Check sheet for the modelled part. Datum: model origin and axes. Units: mm. Face numbers are marked on the shaded views. A direction names the side the tool comes from. Round coordinates to 2 decimals unless told otherwise and drop trailing zeros. Write each loop counter-clockwise with the first axis right and the second up, starting at its lowest first coordinate (ties: lowest second). Pieces come first, ordered by that corner, then holes. Notation, with made-up numbers: (-4.75, 17) - (36.25, 17) arc R15 ccw to (36.25, 22) - close; hole circle Ø11 at (11.5, -11). An arc over 180 degrees is marked (long way). Use one line per item in the form item = value. Start each with the question number.
1) Draft check along X on the marked faces 3, 4 and 5. Enter one of: +X half, -X half, draft (parallel to the pull), parting line (faces both ways), or undercut.
2) Scan lines: probe 1 along Y at (x, z) = (0, 3.95); probe 2 along X at (y, z) = (-2, 1.45); probe 3 along X at (y, z) = (16, 1.05). Record each from-to range of solid material in increasing order.
3) Section check D-D (x = 7.5). Record the boundary of the cut face in (y, z).
4) Gauge pin test, flat ends, axial feed: P1, Ø2, axis at x = -14.5, y = 17, coming from the -Z side; P2, Ø1.5, axis at x = -23, y = 0, coming from the -Z side; P3, Ø1, axis at x = -12.5, z = 3, coming from the +Y side. Record the tip position at first contact, or that the pin passes through.
5) Section check A-A (x = 0). Record the boundary of the cut face in (y, z), then the cut area to 3 significant figures.
6) Set-up check for the marked faces 1 and 2: record each of +Z, -Z, +X, -X, +Y, -Y from which the full face is reachable in a straight line by a thin tool's end or side.
7) Section check C-C (y = 7). Record the boundary of the cut face in (x, z).
from build123d import *

# Parameters (mm, degrees)
SKETCH1_R           = 29
BOSS_EXTRUDE1_DEPTH = 4
SKETCH2_R           = 15
CUT_EXTRUDE1_DEPTH  = 24
SKETCH3_R           = 4
BOSS_EXTRUDE2_DEPTH = 1
SKETCH5_R           = 2.5
CUT_EXTRUDE2_DEPTH  = 4.5
CIRPATTERN1_COUNT   = 4
SKETCH6_R           = 3.5
BOSS_EXTRUDE3_DEPTH = 1
SKETCH7_R           = 3.5
CUT_EXTRUDE3_DEPTH  = 2
SKETCH8_R           = 2.5
CUT_EXTRUDE4_DEPTH  = 10
CIRPATTERN2_COUNT   = 4


with BuildPart() as part:
    # Sketch1 → Boss-Extrude1 (new body)
    with BuildSketch(Plane.XY):
        Circle(SKETCH1_R)
    extrude(amount=BOSS_EXTRUDE1_DEPTH)

    # Sketch2 → Cut-Extrude1 (cut)
    with BuildSketch(Plane.XY.offset(4)):
        Circle(SKETCH2_R)
    extrude(amount=-CUT_EXTRUDE1_DEPTH, mode=Mode.SUBTRACT)

    # Sketch3 → Boss-Extrude2 (add)
    with BuildSketch(Plane.XY.offset(4)):
        with Locations((0, 22)):
            Circle(SKETCH3_R)
    boss_extrude2 = extrude(amount=BOSS_EXTRUDE2_DEPTH)

    # Sketch5 → Cut-Extrude2 (cut)
    with BuildSketch(Plane(origin=(0, 0, 0), x_dir=(-1, 0, 0), z_dir=(0, 0, -1))):
        with Locations((0, 22)):
            Circle(SKETCH5_R)
    cut_extrude2 = extrude(amount=-CUT_EXTRUDE2_DEPTH, mode=Mode.SUBTRACT)

    # CirPattern1: Boss-Extrude2, Cut-Extrude2 ×4 about axis
    cirpattern1_axis = Axis((0, 0, 0), (0, 0, 1))
    add([boss_extrude2.rotate(cirpattern1_axis, i * 360 / CIRPATTERN1_COUNT) for i in range(1, CIRPATTERN1_COUNT)])
    add([cut_extrude2.rotate(cirpattern1_axis, i * 360 / CIRPATTERN1_COUNT) for i in range(1, CIRPATTERN1_COUNT)], mode=Mode.SUBTRACT)

    # Sketch6 → Boss-Extrude3 (add)
    with BuildSketch(Plane.XY.offset(4)):
        with Locations((-15.556349186, 15.556349186)):
            Circle(SKETCH6_R)
    boss_extrude3 = extrude(amount=BOSS_EXTRUDE3_DEPTH)

    # Sketch7 → Cut-Extrude3 (cut)
    with BuildSketch(Plane(origin=(0, 0, 0), x_dir=(-1, 0, 0), z_dir=(0, 0, -1))):
        with Locations(Location((15.556349186, 15.556349186, 0), (0, 0, 180))):
            Circle(SKETCH7_R)
    cut_extrude3 = extrude(amount=-CUT_EXTRUDE3_DEPTH, mode=Mode.SUBTRACT)

    # Sketch8 → Cut-Extrude4 (cut)
    with BuildSketch(Plane(origin=(0, 0, 2), x_dir=(-1, 0, 0), z_dir=(0, 0, -1))):
        with Locations((15.556349186, 15.556349186)):
            Circle(SKETCH8_R)
    cut_extrude4 = extrude(amount=-CUT_EXTRUDE4_DEPTH, mode=Mode.SUBTRACT)

    # CirPattern2: Boss-Extrude3, Cut-Extrude3, Cut-Extrude4 ×4 about axis
    cirpattern2_axis = Axis((0, 0, 0), (0, 0, 1))
    add([boss_extrude3.rotate(cirpattern2_axis, i * 360 / CIRPATTERN2_COUNT) for i in range(1, CIRPATTERN2_COUNT)])
    add([cut_extrude3.rotate(cirpattern2_axis, i * 360 / CIRPATTERN2_COUNT) for i in range(1, CIRPATTERN2_COUNT)], mode=Mode.SUBTRACT)
    add([cut_extrude4.rotate(cirpattern2_axis, i * 360 / CIRPATTERN2_COUNT) for i in range(1, CIRPATTERN2_COUNT)], mode=Mode.SUBTRACT)


solid = part.part
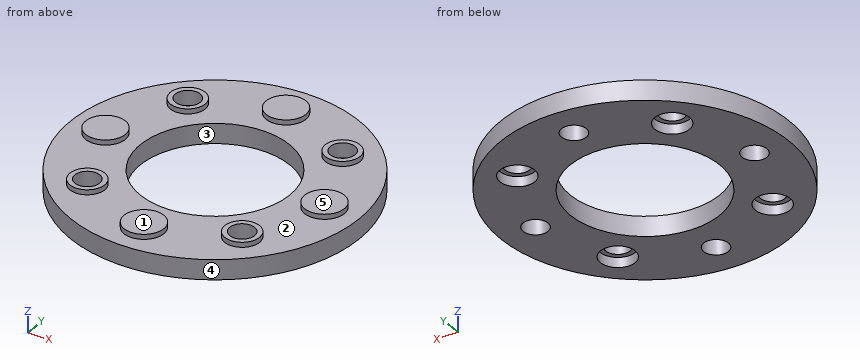
Results are:
q1.face_3 = undercut
q1.face_4 = parting line
q1.face_5 = draft
q2.probe_1 = -29 to -24.5, -19.5 to -15, 15 to 19.5, 24.5 to 29
q2.probe_2 = -28.93 to -23.5, -20.5 to -14.87, 14.87 to 20.5, 23.5 to 28.93
q2.probe_3 = -24.19 to -19.03, -12.08 to 12.08, 19.03 to 24.19
q3.outline = (-28.01, 0) - (-12.99, 0) - (-12.99, 4) - (-28.01, 4) - close; (12.99, 0) - (28.01, 0) - (28.01, 4) - (12.99, 4) - close
q4.P1 = 2
q4.P2 = 4.5
q4.P3 = 26.4
q5.outline = (-29, 0) - (-24.5, 0) - (-24.5, 4.5) - (-19.5, 4.5) - (-19.5, 0) - (-15, 0) - (-15, 4) - (-18, 4) - (-18, 5) - (-26, 5) - (-26, 4) - (-29, 4) - close; (15, 0) - (19.5, 0) - (19.5, 4.5) - (24.5, 4.5) - (24.5, 0) - (29, 0) - (29, 4) - (26, 4) - (26, 5) - (18, 5) - (18, 4) - (15, 4) - close
q5.area = 83.0 mm²
q6.face_1 = +Z, +X, -X, +Y, -Y
q6.face_2 = +Z
q7.outline = (-28.14, 0) - (-13.27, 0) - (-13.27, 4) - (-28.14, 4) - close; (13.27, 0) - (28.14, 0) - (28.14, 4) - (13.27, 4) - close
